Here's the drawing with two shaded views (mm, measured from the low corner). I have some questions. Round coordinates to 2 decimals unless told otherwise and drop trailing zeros. Loops run counter-clockwise (first coordinate to the right, second up) from the corner with the lowest first, then second, coordinate; pieces in that order, holes last.
(1) I want a section at B-B on x = 55. Write out the boundary of the cut face in (y, z), plus the area to 4 significant figures.
(2) I want a section at C-C on y = 0.8. Write out the boundary of the cut face in (x, z), plus the area to 3 significant figures.
(3) If I drill on line 1 along X through (y, z) = (1.3, 15); line 2 along Z through (x, y) = (40, 2.1); line 3 along X through (y, z) = (3.75, 23), over which ranges is the centre line in solid material (lowest first)?
(4) I want a section at A-A on z = 15. Write out the boundary of the cut face in (x, y).
(5) Will this pin go through, and if not, where does the flat tip stop? pin 1 Ø2 at (x, y) = (55, 1.5) entering from +Z.
(6) Thinking about a two-plate mould opening in X: for the marked faces 1, 2 and 3, which applies, released by +X, released by -X, zero draft, split by the parting line, or undercut?
(7) I want a section at D-D on x = 36. Write out the boundary of the cut face in (y, z), plus the area to 3 significant figures.
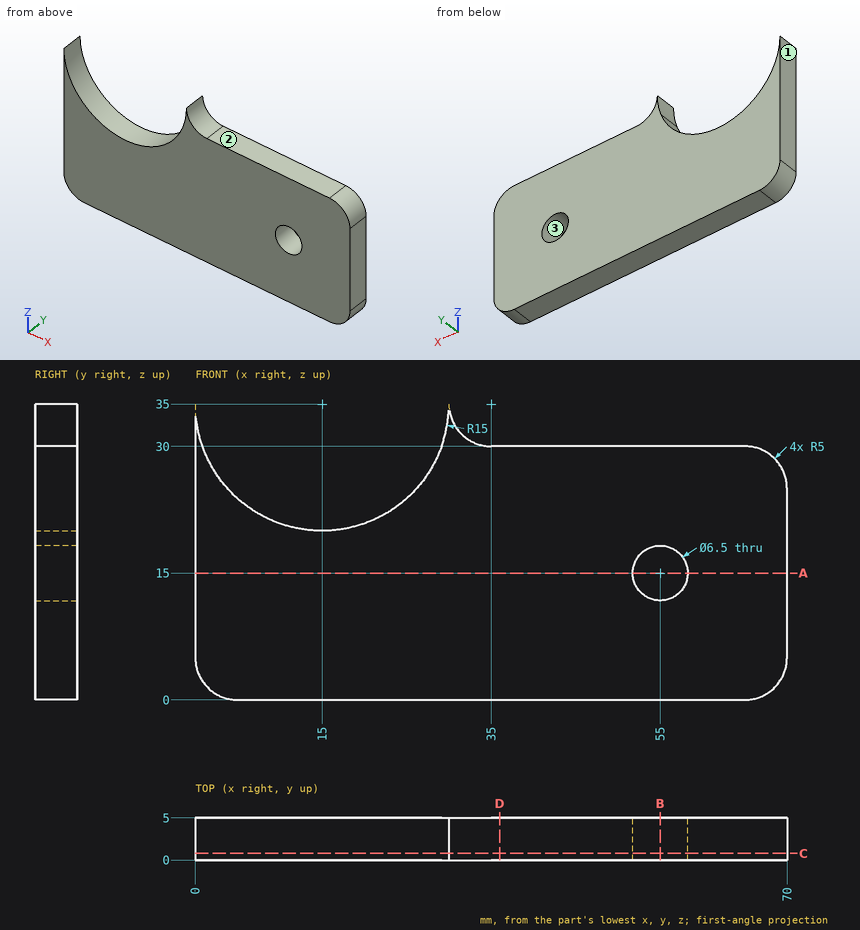
Filled sheet:
1. outline: (0, 0) - (5, 0) - (5, 11.75) - (0, 11.75) - close; (0, 18.25) - (5, 18.25) - (5, 30) - (0, 30) - close
1. area: 117.5 mm2
2. outline: (0, 5) arc R5 ccw to (5, 0) - (65, 0) arc R5 ccw to (70, 5) - (70, 25) arc R5 ccw to (65, 30) - (35, 30) arc R5 cw to (30, 35) arc R15 cw to (0, 35) - close; hole circle Ø6.5 at (55, 15)
2. area: 1,850 mm2
3. line 1: x = 0 to 51.75, 58.25 to 70
3. line 2: z = 0 to 30
3. line 3: x = 0 to 6, 24 to 70
4. outline: (0, 0) - (51.75, 0) - (51.75, 5) - (0, 5) - close; (58.25, 0) - (70, 0) - (70, 5) - (58.25, 5) - close
5. pin 1: stops at z = 30
6. face 1: released by -X
6. face 2: zero draft
6. face 3: undercut
7. outline: (0, 0) - (5, 0) - (5, 30) - (0, 30) - close
7. area: 150 mm2
